CAD build for the part. Positions are in the model's coordinates, mm. Face numbers are marked on the shaded views. A direction names the side the tool comes from. Coordinates: 2 decimals unless noted, no trailing zeros. Write each loop counter-clockwise with the first axis right and the second up, starting at its lowest first coordinate (ties: lowest second). Pieces come first, ordered by that corner, then holes. Notation, with made-up numbers: (7, -37.5) - (29, -37.5) arc R8 cw to (29, -25.5) - close; hole circle Ø4 at (-37, 13.25). An arc over 180 degrees is marked (long way). Answer in a Markdown table with one row per item. Add a question column.
Q1. Band-saw the part on C-C (y = 4). List the corners of the cut face in (x, z).
Q2. Drill centre lines: line 1 along Y through (x, z) = (2, 4.5); line 2 along X through (y, z) = (23.5, -0.5); line 3 along X through (y, z) = (-18, 0). Where is each one in solid material? Low to high. Write a range as from..to.
Q3. 3-axis set-ups, long thin cutter, end or side, ignore diameter. For the marked faces 1, 2 and 3: which of +Z, -Z, +X, -X, +Y, -Y reach the whole face in a straight line?
Q4. Band-saw the part on A-A (z = 0). List the corners of the cut face in (x, y).
Q5. Pin check, flat tips, straight feed: pin 1 (2 mm diameter, centred on x = 3.5, y = -17.5, fed in from -Z); pin 2 (1.5 mm diameter, centred on x = 0, z = 0, fed in from +Y); pin 3 (4 mm diameter, centred on x = 2.5, y = -3, fed in from +Z). Stop position of each tip, or through.
Q6. Band-saw the part on B-B (y = 13). List the corners of the cut face in (x, z).
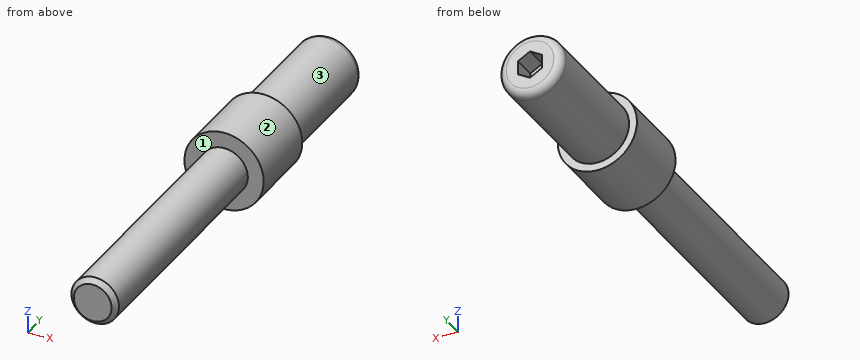
```python
from build123d import *

# Parameters (mm, degrees)
CUT_EXTRUDE_1_DEPTH      = 3
CUT_EXTRUDE_1_DEPTH_BACK = 3


with BuildPart() as part:
    # 草图1 → 旋转1 (revolve)
    with BuildSketch(Plane.XY, mode=Mode.PRIVATE) as revolve_1_sk:
        with BuildLine():
            Line((0, 25.8), (3, 25.8))
            ThreePointArc((3, 25.8), (3.707106781, 25.507106781), (4, 24.8))
            Line((4, 24.8), (4, 9.4))
            Line((4, 9.4), (5, 9.4))
            Line((5, 9.4), (5, 0))
            Line((5, 0), (3, 0))
            Line((3, 0), (3, -31.3865))
            Line((3, -31.3865), (2.3865, -32))
            Line((2.3865, -32), (0, -32))
            Line((0, -32), (0, 25.8))
        make_face()
    revolve(revolve_1_sk.sketch.rotate(Axis((0, -32, 0), (0, 1, 0)), 270), axis=Axis((0, -32, 0), (0, 1, 0)))

    # 草图2 → 切除-拉伸1 (cut, two sides: drawn at the far end of the back side and taken through both)
    with BuildSketch(Plane(origin=(0, 25.8, 0), x_dir=(1, 0, 0), z_dir=(0, 1, 0)).offset(-CUT_EXTRUDE_1_DEPTH_BACK)):
        Polygon((-1.5, 0.866025404), (-1.5, -0.866025404), (0, -1.732050808), (1.5, -0.866025404), (1.5, 0.866025404), (0, 1.732050808), align=None)
    extrude(amount=CUT_EXTRUDE_1_DEPTH + CUT_EXTRUDE_1_DEPTH_BACK, mode=Mode.SUBTRACT)


solid = part.part
```
Checked values:
| question | item | result |
|---|---|---|
| 1 | outline | circle Ø10 at (0, 0) |
| 2 | line 1 | y = 0..9.4 |
| 2 | line 2 | x = -3.97..-1.5, 1.5..3.97 |
| 2 | line 3 | x = -3..3 |
| 3 | face 1 | -Y |
| 3 | face 2 | +Y, -Y |
| 3 | face 3 | +Y |
| 4 | outline | (-5, 0) - (-3, 0) - (-3, -31.39) - (-2.39, -32) - (2.39, -32) - (3, -31.39) - (3, 0) - (5, 0) - (5, 9.4) - (4, 9.4) - (4, 24.8) arc R1 ccw to (3, 25.8) - (1.5, 25.8) - (1.5, 22.8) - (-1.5, 22.8) - (-1.5, 25.8) - (-3, 25.8) arc R1 ccw to (-4, 24.8) - (-4, 9.4) - (-5, 9.4) - close |
| 5 | pin 1 | stops at z = -1.66 |
| 5 | pin 2 | stops at y = 22.8 |
| 5 | pin 3 | stops at z = 2.96 |
| 6 | outline | circle Ø8 at (0, 0) |
